Can you work these out from the drawing? Everything is in mm from the part's minimum corner. A direction names the side the tool comes from. Coordinates: 2 decimals unless noted, no trailing zeros. Loops run counter-clockwise (first coordinate to the right, second up) from the corner with the lowest first, then second, coordinate; pieces in that order, holes last. Notation, with made-up numbers: (69.25, 83.25) -> (107.25, 83.25) arc R25 ccw to (107.25, 112.25) -> close; hole circle Ø1 at (65.5, 58.25). An arc over 180 degrees is marked (long way). One line per question, with ' | ' between items.
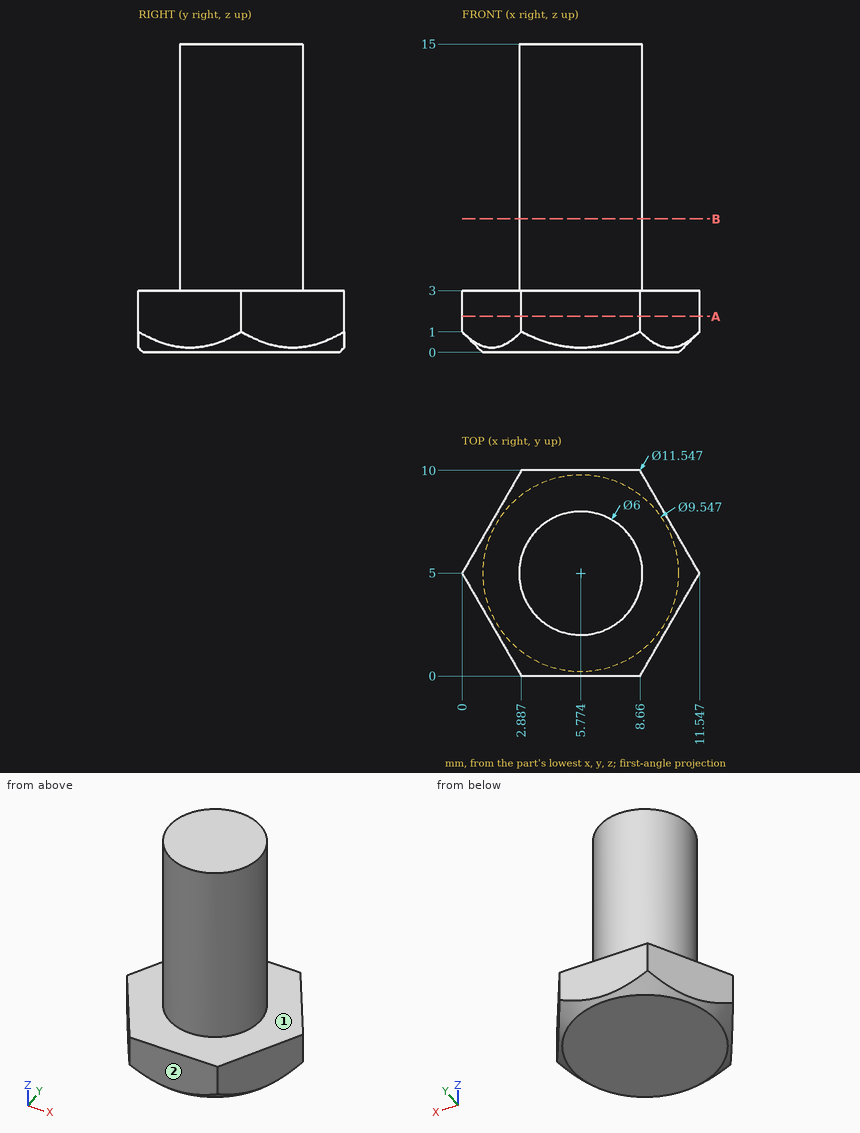
Q1. Imagine slicing it at B-B on z = 6.5. Write out the boundary of the cut face in (x, y), plus the area to 3 significant figures.
Values follow:
outline: circle Ø6 at (5.77, 5) | area: 28.3 mm2
Q2. For pin 1 (1.5 mm diameter, centred on x = 7.5, z = 5.5, fed in from -Y); pin 2 (1.5 mm diameter, centred on y = 7.5, z = 4.5, fed in from +X); pin 3 (4 mm diameter, centred on y = 2.5, z = 13.5, fed in from -X) (1 decimal), each with a flat end and sliding along its axis, tell me the tip position at first contact or that it passes through.
Values follow:
pin 1: stops at y = 2.16 | pin 2: stops at x = 8.21 | pin 3: stops at x = 2.8
Q3. Please list where these lines run through material, in increasing order: L1, parallel to Z at x = 2.5, y = 5.75; L2, parallel to Z at x = 10.75, y = 4.5; L3, parallel to X at y = 7.5, z = 3.5 (1 decimal). Write a range as [from, to].
Values follow:
L1: z = [0, 3] | L2: z = [0.23, 3] | L3: x = [4.1, 7.4]
Q4. For the marked faces 1 and 2, which set-ups out of +Z, -Z, +X, -X, +Y, -Y let a thin tool reach every point of the face, with its end or its side?
Values follow:
face 1: +Z | face 2: +Z, -Z, +X, -X, -Y
Q5. Imagine slicing it at A-A on z = 1.75. Write out the boundary of the cut face in (x, y), plus the area to 3 significant figures.
Values follow:
outline: (0, 5) -> (2.89, 0) -> (8.66, 0) -> (11.55, 5) -> (8.66, 10) -> (2.89, 10) -> close | area: 86.6 mm2
